```python
from build123d import *

# Parameters (mm, degrees)
FLANGE_SKETCH_R                   = 44.45
FLANGE_3_5_DEPTH                  = 12.7
HUB_BOSS_SKETCH_R                 = 25.4
HUB_BOSS_2_DEPTH                  = 50.8
REAR_RECESS_SKETCH_R              = 20.6375
REAR_RECESS_1_625_DEPTH           = 6.35
PILOT_BORE_SKETCH_R               = 9.525
PILOT_BORE_0_75_DEPTH             = 9.525
INNER_BORE_SKETCH_R               = 12.7
INNER_BORE_1_0_DEPTH              = 25.4
BEARING_BORE_SKETCH_R             = 14.2875
BEARING_BORE_1_125_DEPTH          = 15.875
RETAINING_GROOVE_SKETCH_R         = 15.8115
RETAINING_RING_GROOVE_1_245_DEPTH = 1.143
THROUGH_BORE_SKETCH_R             = 14.2875
THROUGH_BORE_1_125_DEPTH          = 86.730267986
BOLT_COUNTERBORE_SKETCH_R         = 5.1562
BOLT_COUNTERBORES_6X_0_406_DEPTH  = 6.35
BOLT_HOLE_SKETCH_R                = 3.5687
BOLT_HOLES_6X_0_281_DEPTH         = 85.957209818
HUB_ROOT_FILLET_R0_125_R          = 3.175


with BuildPart() as part:
    # Flange Sketch → Flange Ø3.5 (new body)
    with BuildSketch(Plane.XY):
        Circle(FLANGE_SKETCH_R)
    extrude(amount=FLANGE_3_5_DEPTH)

    # Hub Boss Sketch → Hub Boss Ø2 (add)
    with BuildSketch(Plane.XY.offset(12.7)):
        Circle(HUB_BOSS_SKETCH_R)
    extrude(amount=HUB_BOSS_2_DEPTH)

    # Rear Recess Sketch → Rear Recess Ø1.625 (cut)
    with BuildSketch(Plane(origin=(0, 0, 0), x_dir=(-1, 0, 0), z_dir=(0, 0, -1))):
        Circle(REAR_RECESS_SKETCH_R)
    extrude(amount=-REAR_RECESS_1_625_DEPTH, mode=Mode.SUBTRACT)

    # Pilot Bore Sketch → Pilot Bore Ø0.75 (cut)
    with BuildSketch(Plane(origin=(0, 0, 6.35), x_dir=(-1, 0, 0), z_dir=(0, 0, -1))):
        Circle(PILOT_BORE_SKETCH_R)
    extrude(amount=-PILOT_BORE_0_75_DEPTH, mode=Mode.SUBTRACT)

    # Inner Bore Sketch → Inner Bore Ø1.0 (cut)
    with BuildSketch(Plane(origin=(0, 0, 15.875), x_dir=(-1, 0, 0), z_dir=(0, 0, -1))):
        Circle(INNER_BORE_SKETCH_R)
    extrude(amount=-INNER_BORE_1_0_DEPTH, mode=Mode.SUBTRACT)

    # Bearing Bore Sketch → Bearing Bore Ø1.125 (cut)
    with BuildSketch(Plane(origin=(0, 0, 41.275), x_dir=(-1, 0, 0), z_dir=(0, 0, -1))):
        Circle(BEARING_BORE_SKETCH_R)
    extrude(amount=-BEARING_BORE_1_125_DEPTH, mode=Mode.SUBTRACT)

    # Retaining Groove Sketch → Retaining Ring Groove Ø1.245 (cut)
    with BuildSketch(Plane(origin=(0, 0, 57.15), x_dir=(-1, 0, 0), z_dir=(0, 0, -1))):
        Circle(RETAINING_GROOVE_SKETCH_R)
    extrude(amount=-RETAINING_RING_GROOVE_1_245_DEPTH, mode=Mode.SUBTRACT)

    # Through Bore Sketch → Through Bore Ø1.125 (cut, through all)
    with BuildSketch(Plane(origin=(0, 0, 58.293), x_dir=(-1, 0, 0), z_dir=(0, 0, -1))):
        Circle(THROUGH_BORE_SKETCH_R)
    extrude(amount=-THROUGH_BORE_1_125_DEPTH, mode=Mode.SUBTRACT)

    # Bolt Counterbore Sketch → Bolt Counterbores 6xØ0.406 (cut)
    with BuildSketch(Plane(origin=(0, 0, 0), x_dir=(-1, 0, 0), z_dir=(0, 0, -1))):
        with Locations((0, 38.345083234)):
            Circle(BOLT_COUNTERBORE_SKETCH_R)
        with Locations((33.207816191, 19.172541617)):
            Circle(BOLT_COUNTERBORE_SKETCH_R)
        with Locations((33.207816191, -19.172541617)):
            Circle(BOLT_COUNTERBORE_SKETCH_R)
        with Locations((0, -38.345083234)):
            Circle(BOLT_COUNTERBORE_SKETCH_R)
        with Locations((-33.207816191, -19.172541617)):
            Circle(BOLT_COUNTERBORE_SKETCH_R)
        with Locations((-33.207816191, 19.172541617)):
            Circle(BOLT_COUNTERBORE_SKETCH_R)
    extrude(amount=-BOLT_COUNTERBORES_6X_0_406_DEPTH, mode=Mode.SUBTRACT)

    # Bolt Hole Sketch → Bolt Holes 6xØ0.281 (cut, through all)
    with BuildSketch(Plane(origin=(0, 0, 6.35), x_dir=(-1, 0, 0), z_dir=(0, 0, -1))):
        with Locations((0, 38.345083234)):
            Circle(BOLT_HOLE_SKETCH_R)
        with Locations((33.207816191, 19.172541617)):
            Circle(BOLT_HOLE_SKETCH_R)
        with Locations((33.207816191, -19.172541617)):
            Circle(BOLT_HOLE_SKETCH_R)
        with Locations((0, -38.345083234)):
            Circle(BOLT_HOLE_SKETCH_R)
        with Locations((-33.207816191, -19.172541617)):
            Circle(BOLT_HOLE_SKETCH_R)
        with Locations((-33.207816191, 19.172541617)):
            Circle(BOLT_HOLE_SKETCH_R)
    extrude(amount=-BOLT_HOLES_6X_0_281_DEPTH, mode=Mode.SUBTRACT)

    # Hub Root Fillet R0.125
    hub_root_fillet_r0_125_edges = [part.edges().sort_by_distance(p)[0] for p in [
        (-25.4, 0, 12.7),
    ]]
    fillet(hub_root_fillet_r0_125_edges, radius=HUB_ROOT_FILLET_R0_125_R)


solid = part.part
```
Verification items for the finished model (mm, model axes). A direction names the side the tool comes from. Give positions to 0.01 mm unless a question says otherwise; leave off trailing zeros. Order: outer loops, then holes, each group sorted by start corner. A loop starts at its lowest first (then second) coordinate and runs counter-clockwise, first axis right, second up. Notation, with made-up numbers: M 31,71 L 35,71 A8 cw 35,86 Z; hole C -31.5,8 d1. An arc over 180 degrees is marked long. Answer in a Markdown table with one row per item. Add a question column.
Item 1: Gauge pin test, flat ends, axial feed: pin 1 (20.5 mm diameter, centred on x = 0, y = 0, fed in from +Z) (3 decimals); pin 2 (16.5 mm diameter, centred on x = -33.21, y = 19.17, fed in from +Z); pin 3 (12 mm diameter, centred on x = -10, z = 12.5, fed in from -Y). Record the tip position at first contact, or that the pin passes through.
Item 2: Tool access check on faces 1 (the flat face through (-5, 9, 15.875)), 2 (the cylindrical face through (12.55, -9.62, 57.71)), 3 (the cylindrical face through (37.3, 16.035, 3.131)), 4 (the cylindrical face through (36.773, -19.016, 9.481)). Record the directions out of +Z, -Z, +X, -X, +Y, -Y that give a thin tool (end or side, any length) a straight path to the whole face; none if there is none.
Item 3: Section check C-C, the plane z = 37. Enter the section's corners in (x, y), and give its area (3 significant figures).
Item 4: Scan lines: probe 1 along Y at (x, z) = (0, 3); probe 2 along Z at (x, y) = (-13, 9.5); probe 3 along X at (y, z) = (4.5, 19). Record each from-to range of solid material in increasing order. Write a range as from..to.
Item 5: Section check D-D, the plane z = 46. Enter the section's corners in (x, y) (1 decimal), and give its area (3 significant figures).
Item 6: Section check B-B, the plane x = 0. State how many separate pieces and enclosed holes the cut face has, and give its area (3 significant figures).
Item 7: Mould release check, pull along Y, two halves, no side actions. Record for faces 5 (the cylindrical face through (0.77, 34.86, 9.48)), 6 (the flat face through (-9, -4, 6.35)), 7 (the cylindrical face through (42.397, 13.352, 6.261)): released by +Y, released by -Y, zero draft, split by the parting line, or undercut.
Filled sheet:
| question | item | result |
|---|---|---|
| 1 | pin 1 | stops at z = 15.875 |
| 1 | pin 2 | stops at z = 12.7 |
| 1 | pin 3 | stops at y = -44.27 |
| 2 | face 1 | +Z |
| 2 | face 2 | none |
| 2 | face 3 | -Z |
| 2 | face 4 | +Z, -Z |
| 3 | outline | C 0,0 d50.8; hole C 0,0 d25.4 |
| 3 | area | 1,520 mm^2 |
| 4 | probe 1 | y = -44.45..-43.5, -33.19..-20.64, 20.64..33.19, 43.5..44.45 |
| 4 | probe 2 | z = 6.35..63.5 |
| 4 | probe 3 | x = -25..-11.88, 11.88..25 |
| 5 | outline | C 0,0 d50.8; hole C 0,0 d28.6 |
| 5 | area | 1,390 mm^2 |
| 6 | separate pieces | 4 |
| 6 | enclosed holes | 0 |
| 6 | area | 1,770 mm^2 |
| 7 | face 5 | undercut |
| 7 | face 6 | undercut |
| 7 | face 7 | split by the parting line |
